Can you work these out from the model? Positions are in its coordinate system, mm. Face numbers are marked on the shaded views. A direction names the side the tool comes from. Coordinates: 2 decimals unless noted, no trailing zeros. Order: outer loops, then holes, each group sorted by start corner. A loop starts at its lowest first (then second) coordinate and runs counter-clockwise, first axis right, second up. Notation, with made-up numbers: (-12.75, -33.5) - (7.25, -33.5) arc R17 ccw to (7.25, -5.5) - close; hole circle Ø5 at (60, 8). An arc over 180 degrees is marked (long way). Return JSON: item names as keys, results as strings. Group by question number.
1) Imagine slicing it at B-B (z = 12.25). Write out the boundary of the cut face in (x, y), and give its area (3 significant figures).
2) Imagine slicing it at A-A (x = 0). Write out the boundary of the cut face in (y, z).
3) If we mould it in two halves opening along X, with no side actions, what happens to the marked faces 3, 4 and 5? For each: pulls with the +X half, pulls with the -X half, needs draft (parallel to the pull), parting line crosses it, or undercut.
4) For pin 1 Ø3 at (x, y) = (-21, -25.5) entering from +Z; pin 2 Ø1 at (x, z) = (-35.5, 15) entering from +Y; pin 3 Ø1.5 at (x, z) = (32.5, 11.5) entering from -Y, each with a flat end and sliding along its axis, tell me the tip position at first contact or that it passes through.
5) Which directions (+Z, -Z, +X, -X, +Y, -Y) give clear straight access to the entire face, cutting with the end or side of a thin tool? Please do the marked faces 1 and 2.
6) If I drill on line 1 along Z through (x, y) = (-6.5, -14.5); line 2 along Y through (x, z) = (0, 9); line 3 along Y through (x, z) = (34.5, 10.5), over which ranges is the centre line in solid material (lowest first)?
7) Imagine slicing it at C-C (y = 20). Write out the boundary of the cut face in (x, z), and give its area (3 significant figures).
```python
from build123d import *

# Parameters (mm, degrees)
BASE_PLATE_DEPTH               = 3
OFFSET_STEP_DEPTH              = 3
STANDOFF_BOSS_PROFILE_3X_16_R  = 8
STANDOFF_BOSSES_3X_16_DEPTH    = 12
MOUNTING_HOLE_PROFILE_3X_6_6_R = 3.3
MOUNTING_HOLES_3X_6_6_DEPTH    = 66


with BuildPart() as part:
    # Base Plate Profile → Base Plate (new body)
    with BuildSketch(Plane.XY):
        with BuildLine():
            ThreePointArc((42.912667435, -2.73915564), (37.856365651, 20.393518081), (21.320581008, 37.342105263))
            ThreePointArc((21.320581008, 37.342105263), (17.024750702, 41.150119272), (14.618361477, 46.362068966))
            ThreePointArc((14.618361477, 46.362068966), (-1.031761946, 57.964473505), (-14.941453584, 44.323995772))
            ThreePointArc((-14.941453584, 44.323995772), (-16.147655157, 40.973517523), (-18.846153454, 38.65))
            ThreePointArc((-18.846153454, 38.65), (-37.385977476, 21.243556391), (-42.849619055, -3.593069277))
            ThreePointArc((-42.849619055, -3.593069277), (-43.464441702, -7.100578343), (-45.725338247, -9.851755099))
            ThreePointArc((-45.725338247, -9.851755099), (-49.826116824, -29.687675595), (-30.429578698, -35.523293437))
            ThreePointArc((-30.429578698, -35.523293437), (-26.93387798, -34.844542215), (-23.556567678, -35.9734363))
            ThreePointArc((-23.556567678, -35.9734363), (0.447275802, -42.997673709), (24.299804013, -35.47561874))
            ThreePointArc((24.299804013, -35.47561874), (27.620379782, -34.279599541), (31.102436465, -34.855764987))
            ThreePointArc((31.102436465, -34.855764987), (50.242522242, -28.566226035), (45.85893495, -8.901909464))
            ThreePointArc((45.85893495, -8.901909464), (43.583057713, -6.204305311), (42.912667435, -2.73915564))
        make_face()
    extrude(amount=BASE_PLATE_DEPTH)

    # Offset Step Profile → Offset Step (add)
    with BuildSketch(Plane.XY.offset(3)):
        with BuildLine():
            ThreePointArc((-17.531305538, 35.953488372), (-34.777653466, 19.761447806), (-39.860110749, -3.342390025))
            ThreePointArc((-39.860110749, -3.342390025), (-40.738428815, -8.353117262), (-43.968281023, -12.283369771))
            ThreePointArc((-43.968281023, -12.283369771), (-47.248903885, -28.152106168), (-31.731673384, -32.820600441))
            ThreePointArc((-31.731673384, -32.820600441), (-26.737815215, -31.850955839), (-21.913086212, -33.463661675))
            ThreePointArc((-21.913086212, -33.463661675), (0.416070514, -39.997836008), (22.604468849, -33.000575572))
            ThreePointArc((22.604468849, -33.000575572), (27.34814852, -31.291976717), (32.32251521, -32.11507021))
            ThreePointArc((32.32251521, -32.11507021), (47.634583832, -27.083439049), (44.127713998, -11.351985792))
            ThreePointArc((44.127713998, -11.351985792), (40.876460802, -7.498265573), (39.918760405, -2.548051758))
            ThreePointArc((39.918760405, -2.548051758), (35.215223861, 18.970714494), (19.833098612, 34.736842105))
            ThreePointArc((19.833098612, 34.736842105), (14.616733241, 39.360859116), (11.694689182, 45.689655172))
            ThreePointArc((11.694689182, 45.689655172), (-0.825409557, 54.971578804), (-11.953162867, 44.059196617))
            ThreePointArc((-11.953162867, 44.059196617), (-13.676307972, 39.272799119), (-17.531305538, 35.953488372))
        make_face()
    extrude(amount=OFFSET_STEP_DEPTH)

    # Standoff Boss Profile 3xØ16 → Standoff Bosses 3xØ16 (add)
    with BuildSketch(Plane.XY.offset(6)):
        with Locations((0, 43)):
            Circle(STANDOFF_BOSS_PROFILE_3X_16_R)
        with Locations((37.202830189, -21.152291105)):
            Circle(STANDOFF_BOSS_PROFILE_3X_16_R)
        with Locations((-36.940052128, -22.009828458)):
            Circle(STANDOFF_BOSS_PROFILE_3X_16_R)
    extrude(amount=STANDOFF_BOSSES_3X_16_DEPTH)

    # Mounting Hole Profile 3xØ6.6 → Mounting Holes 3xØ6.6 (cut)
    with BuildSketch(Plane.XY.offset(18)):
        with Locations((0, 43)):
            Circle(MOUNTING_HOLE_PROFILE_3X_6_6_R)
        with Locations((37.202830189, -21.152291105)):
            Circle(MOUNTING_HOLE_PROFILE_3X_6_6_R)
        with Locations((-36.940052128, -22.009828458)):
            Circle(MOUNTING_HOLE_PROFILE_3X_6_6_R)
    extrude(amount=-MOUNTING_HOLES_3X_6_6_DEPTH, mode=Mode.SUBTRACT)


solid = part.part
```
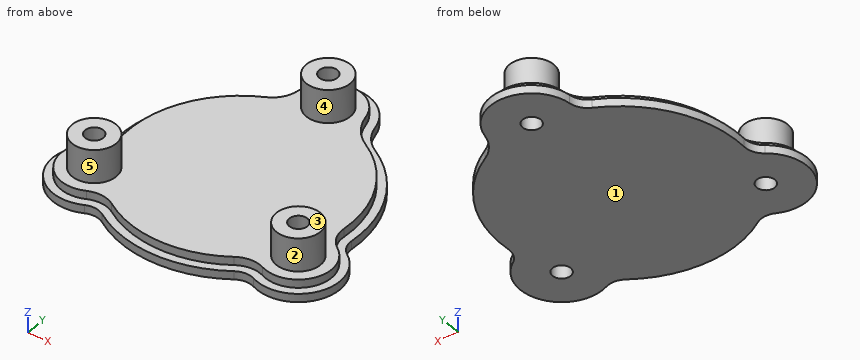
Calculated:
{
 "1": {"outline": "circle Ø16 at (-36.94, -22.01); circle Ø16 at (0, 43); circle Ø16 at (37.2, -21.15); hole circle Ø6.6 at (-36.94, -22.01); hole circle Ø6.6 at (0, 43); hole circle Ø6.6 at (37.2, -21.15)", "area": "501 mm2"},
 "2": {"outline": "(-43, 0) - (39.7, 0) - (39.7, 18) - (35, 18) - (35, 6) - (-40, 6) - (-40, 3) - (-43, 3) - close; (46.3, 0) - (58, 0) - (58, 3) - (55, 3) - (55, 6) - (51, 6) - (51, 18) - (46.3, 18) - close"},
 "3": {"face 3": "needs draft", "face 4": "parting line crosses it", "face 5": "undercut"},
 "4": {"pin 1": "z = 6", "pin 2": "y = -14.07", "pin 3": "y = -28.11"},
 "5": {"face 1": "-Z, +X, -X, +Y, -Y", "face 2": "+Z"},
 "6": {"line 1": "0 to 6", "line 2": "35 to 39.7, 46.3 to 51", "line 3": "-28.68 to -23.05, -19.26 to -13.62"},
 "7": {"outline": "(-38.07, 0) - (38.07, 0) - (38.07, 3) - (34.64, 3) - (34.64, 6) - (-34.64, 6) - (-34.64, 3) - (-38.07, 3) - close", "area": "436 mm2"}
}
